Part model, mm, in its own coordinate system. Face numbers are marked on the shaded views. A direction names the side the tool comes from. Round coordinates to 2 decimals unless told otherwise and drop trailing zeros. Loops run counter-clockwise (first coordinate to the right, second up) from the corner with the lowest first, then second, coordinate; pieces in that order, holes last. Notation, with made-up numbers: M 80.25,-8.75 L 94.25,-8.75 A11 ccw 94.25,-2.75 Z; hole C 41.25,44 d2. An arc over 180 degrees is marked long. Put each result on its own line as item: value. Start each with the question number.
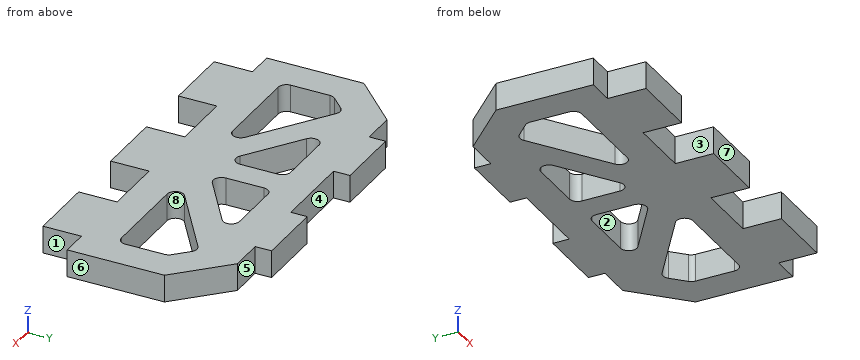
```python
from build123d import *

# Parameters (mm, degrees)
EXTRUDE_1_DEPTH = 5
FILLET_3_R      = 1.5
FILLET_4_R      = 1.5
FILLET_5_R      = 1.5


with BuildPart() as part:
    # 草图1 → 凸台-拉伸1 (new body)
    with BuildSketch(Plane.XY):
        Polygon((7.785235828, 15.309450129), (-7.214764172, 15.309450129), (-7.214764172, 18.309450129), (-19.714764172, 18.309450129), (-19.714764172, 15.309450129), (-25.964764172, 15.309450129), (-34.714764172, 6.559450129), (-34.714764172, -11.190549871), (-29.714764172, -11.190549871), (-29.714764172, -18.207876603), (-17.214764172, -18.207876603), (-17.214764172, -11.190549871), (-5.964764172, -11.190549871), (-5.964764172, -18.207876603), (6.535235828, -18.207876603), (6.535235828, -11.190549871), (17.785235828, -11.190549871), (17.785235828, -18.207876603), (30.285235828, -18.207876603), (30.285235828, -11.190549871), (35.285235828, -11.190549871), (35.285235828, 6.559450129), (26.535235828, 15.309450129), (20.285235828, 15.309450129), (20.285235828, 18.309450129), (7.785235828, 18.309450129), align=None)
        Polygon((-24.987626131, 7.801306796), (-28.714764172, 4.074168755), (-28.714764172, -5.190549871), (-6.433331929, -5.190549871), align=None, mode=Mode.SUBTRACT)
        Polygon((-18.424244048, 9.309450129), (-2.214764172, 9.309450129), (-2.214764172, -2.040549871), align=None, mode=Mode.SUBTRACT)
        Polygon((2.785235828, -2.040549871), (18.994715705, 9.309450129), (2.785235828, 9.309450129), align=None, mode=Mode.SUBTRACT)
        Polygon((7.003803585, -5.190549871), (25.558097787, 7.801306796), (29.285235828, 4.074168755), (29.285235828, -5.190549871), align=None, mode=Mode.SUBTRACT)
    extrude(amount=EXTRUDE_1_DEPTH)

    # 圆角3
    fillet_3_edges = [part.edges().sort_by_distance(p)[0] for p in [
        (-24.987626131, 7.801306796, 2.5),
    ]]
    fillet(fillet_3_edges, radius=FILLET_3_R)

    # 圆角4
    fillet_4_edges = [part.edges().sort_by_distance(p)[0] for p in [
        (-6.433331929, -5.190549871, 2.5),
        (-28.714764172, 4.074168755, 2.5),
        (-28.714764172, -5.190549871, 2.5),
    ]]
    fillet(fillet_4_edges, radius=FILLET_4_R)

    # 圆角5
    fillet_5_edges = [part.edges().sort_by_distance(p)[0] for p in [
        (29.285235828, -5.190549871, 2.5),
        (29.285235828, 4.074168755, 2.5),
        (25.558097787, 7.801306796, 2.5),
        (-18.424244048, 9.309450129, 2.5),
        (-2.214764172, -2.040549871, 2.5),
        (-2.214764172, 9.309450129, 2.5),
        (2.785235828, 9.309450129, 2.5),
        (2.785235828, -2.040549871, 2.5),
        (18.994715705, 9.309450129, 2.5),
        (7.003803585, -5.190549871, 2.5),
    ]]
    fillet(fillet_5_edges, radius=FILLET_5_R)


solid = part.part
```
1. Cut at B-B, the plane y = 2. Give the cut face in (x, z), and give its area (3 significant figures).
2. Cut at A-A, the plane x = 22.5. Give the cut face in (y, z).
3. Cut at D-D, the plane y = 11. Give the cut face in (x, z).
4. Wall check: L1, parallel to X at y = -12.5, z = 3.8; L2, parallel to X at y = 1.5, z = 1.95; L3, parallel to Y at x = -14.5, z = 2.9. Give the ranges that are in metal, low to high.
5. Which spindle directions (+Z, -Z, +X, -X, +Y, -Y) get a long thin tool onto all of the face, cutting with end or side? Do the marked faces 1, 2, 3, 4 and 5. Say none if no direction does.
6. Mould opens along Y. For the marked faces 6, 7 and 8 say: released by +Y, released by -Y, zero draft, split by the parting line, or undercut.
7. Drop flat-ended pins along their axis: pin 1 (1.5 mm diameter, centred on y = -14, z = 3, fed in from -X); pin 2 (1.5 mm diameter, centred on x = -24.5, z = 3, fed in from +Y); pin 3 (1.5 mm diameter, centred on y = -14, z = 2.5, fed in from +X). Give the stop position or say it passes through.
8. Cut at C-C, the plane z = 0.9. Give the number of separate pieces and of enclosed holes in the cut face, and give its area (3 significant figures).
Results list:
1. outline: M -34.71,0 L -28.71,0 L -28.71,5 L -34.71,5 Z; M -16.7,0 L -7.99,0 L -7.99,5 L -16.7,5 Z; M -2.21,0 L 2.79,0 L 2.79,5 L -2.21,5 Z; M 8.56,0 L 17.27,0 L 17.27,5 L 8.56,5 Z; M 29.29,0 L 35.29,0 L 35.29,5 L 29.29,5 Z
1. area: 172 mm^2
2. outline: M -18.21,0 L -5.19,0 L -5.19,5 L -18.21,5 Z; M 5.66,0 L 15.31,0 L 15.31,5 L 5.66,5 Z
3. outline: M -30.27,0 L 30.84,0 L 30.84,5 L -30.27,5 Z
4. L1: x = -29.71 to -17.21, -5.96 to 6.54, 17.79 to 30.29
4. L2: x = -34.71 to -28.71, -15.99 to -7.27, -2.21 to 2.79, 7.84 to 16.56, 29.29 to 35.29
4. L3: y = -11.19 to -5.19, 0.46 to 6.56, 9.06 to 18.31
5. face 1: +Z, -Z, +X, -Y
5. face 2: +Z, -Z
5. face 3: +Z, -Z, -Y
5. face 4: +Z, -Z, +Y
5. face 5: +Z, -Z, +X, +Y
6. face 6: zero draft
6. face 7: released by -Y
6. face 8: undercut
7. pin 1: stops at x = -29.71
7. pin 2: stops at y = 15.31
7. pin 3: stops at x = 30.29
8. separate pieces: 1
8. enclosed holes: 4
8. area: 1,630 mm^2
